Design review of the part built by this model. Coordinates are the model's own, in mm. A direction names the side the tool comes from. Coordinates: 2 decimals unless noted, no trailing zeros. Write each loop counter-clockwise with the first axis right and the second up, starting at its lowest first coordinate (ties: lowest second). Pieces come first, ordered by that corner, then holes. Notation, with made-up numbers: (-10, 86.5) - (1, 86.5) arc R10 ccw to (1, 91.5) - close; hole circle Ø9 at (70.5, 71). An arc over 180 degrees is marked (long way). Use a Markdown table: item, result.
from build123d import *

# Parameters (mm, degrees)
SKETCH1_R                = 205
SKETCH1_R_2              = 5
SKETCH1_R_3              = 175
BOSS_EXTRUDE1_DEPTH      = 2
BOSS_EXTRUDE2_DEPTH      = 7
BOSS_EXTRUDE2_DEPTH_BACK = 2
SKETCH2_R                = 207
SKETCH2_R_2              = 205
BOSS_EXTRUDE3_START      = 2
SKETCH3_R                = 207
SKETCH3_R_2              = 195
BOSS_EXTRUDE3_DEPTH      = 2


with BuildPart() as part:
    # Sketch1 → Boss-Extrude1 (new body)
    with BuildSketch(Plane(origin=(0, 0, 0), x_dir=(1, 0, 0), z_dir=(0, 1, 0))):
        with Locations(Location((0, 0, 0), (0, 0, 270))):
            Circle(SKETCH1_R)
        with Locations(Location((-185, 0, 0), (0, 0, 270))):
            Circle(SKETCH1_R_2, mode=Mode.SUBTRACT)
        with Locations(Location((0, 0, 0), (0, 0, 270))):
            Circle(SKETCH1_R_3, mode=Mode.SUBTRACT)
        with Locations(Location((-130.81475452, 130.81475452, 0), (0, 0, 270))):
            Circle(SKETCH1_R_2, mode=Mode.SUBTRACT)
        with Locations(Location((0, 185, 0), (0, 0, 270))):
            Circle(SKETCH1_R_2, mode=Mode.SUBTRACT)
        with Locations(Location((130.81475452, 130.81475452, 0), (0, 0, 270))):
            Circle(SKETCH1_R_2, mode=Mode.SUBTRACT)
        with Locations(Location((185, 0, 0), (0, 0, 270))):
            Circle(SKETCH1_R_2, mode=Mode.SUBTRACT)
        with Locations(Location((130.81475452, -130.81475452, 0), (0, 0, 270))):
            Circle(SKETCH1_R_2, mode=Mode.SUBTRACT)
        with Locations(Location((0, -185, 0), (0, 0, 270))):
            Circle(SKETCH1_R_2, mode=Mode.SUBTRACT)
        with Locations(Location((-130.81475452, -130.81475452, 0), (0, 0, 270))):
            Circle(SKETCH1_R_2, mode=Mode.SUBTRACT)
    extrude(amount=BOSS_EXTRUDE1_DEPTH)

    # Sketch2 → Boss-Extrude2 (add, two sides: drawn at the far end of the back side and taken through both)
    with BuildSketch(Plane.XZ.offset(-BOSS_EXTRUDE2_DEPTH_BACK)):
        with Locations(Location((0, 0, 0), (0, 0, 270))):
            Circle(SKETCH2_R)
        with Locations(Location((0, 0, 0), (0, 0, 270))):
            Circle(SKETCH2_R_2, mode=Mode.SUBTRACT)
    extrude(amount=BOSS_EXTRUDE2_DEPTH + BOSS_EXTRUDE2_DEPTH_BACK)

    # Sketch3 → Boss-Extrude3 (add)
    with BuildSketch(Plane.XZ.offset(7).offset(BOSS_EXTRUDE3_START)):
        with Locations(Location((0, 0, 0), (0, 0, 270))):
            Circle(SKETCH3_R)
        with Locations(Location((0, 0, 0), (0, 0, 270))):
            Circle(SKETCH3_R_2, mode=Mode.SUBTRACT)
    extrude(amount=-BOSS_EXTRUDE3_DEPTH)


solid = part.part
(1) Take a section at B-B on z = 0. Write out the cut boundary in (x, y), and give its area (3 significant figures).
Determined:
| item | result |
|---|---|
| outline | (-207, -9) - (-195, -9) - (-195, -7) - (-205, -7) - (-205, 0) - (-190, 0) - (-190, 2) - (-207, 2) - close; (-180, 0) - (-175, 0) - (-175, 2) - (-180, 2) - close; (175, 0) - (180, 0) - (180, 2) - (175, 2) - close; (190, 0) - (205, 0) - (205, -7) - (195, -7) - (195, -9) - (207, -9) - (207, 2) - (190, 2) - close |
| area | 164 mm2 |
(2) Machinability: for faces 5 (the cylindrical face through (189.957, 0.986, -0.651)), 6 (the flat face through (-75, -7, -181)), 7 (the cylindrical face through (-173, -8.01, -89.98)), which of the approach directions +Z, -Z, +X, -X, +Y, -Y give a long, thin tool a straight path to every point of the face, cutting with its end or side? Answer none if there is none.
Determined:
| item | result |
|---|---|
| face 5 | +Y, -Y |
| face 6 | none |
| face 7 | -Y |
(3) For L1, parallel to X at y = 0.85, z = 0; L2, parallel to Z at x = 6, y = -2.5; L3, parallel to Z at x = -122, y = -3.5, list the stretches that pass through material, from the lowest coordinate up. Write a range as from..to.
Determined:
| item | result |
|---|---|
| L1 | -207..-190, -180..-175, 175..180, 190..207 |
| L2 | -206.91..-204.91, 204.91..206.91 |
| L3 | -167.23..-164.75, 164.75..167.23 |
(4) Take a section at D-D on y = -3.5. Write out the cut boundary in (x, z).
Determined:
| item | result |
|---|---|
| outline | circle Ø414 at (0, 0); hole circle Ø410 at (0, 0) |
(5) Take a section at A-A on x = 0. Write out the cut boundary in (y, z).
Determined:
| item | result |
|---|---|
| outline | (-9, -207) - (2, -207) - (2, -190) - (0, -190) - (0, -205) - (-7, -205) - (-7, -195) - (-9, -195) - close; (-9, 195) - (-7, 195) - (-7, 205) - (0, 205) - (0, 190) - (2, 190) - (2, 207) - (-9, 207) - close; (0, -180) - (2, -180) - (2, -175) - (0, -175) - close; (0, 175) - (2, 175) - (2, 180) - (0, 180) - close |
(6) Draft analysis for pull direction Y (two halves, no side actions). For faces 1 (the cylindrical face through (-130.59, 0.99, -135.81)), 2 (the flat face through (-151, 0, 90)), 3 (the flat face through (-137, -9, 139)), 4 (the cylindrical face through (-200.125, -3.451, 44.44)), state which applies: +Y half, -Y half, draft (parallel to the pull), parting line (faces both ways), or undercut.
Determined:
| item | result |
|---|---|
| face 1 | draft |
| face 2 | undercut |
| face 3 | -Y half |
| face 4 | undercut |
(7) For pin 1 (9 mm diameter, centred on x = 185, z = 0, fed in from +Y); pin 2 (4 mm diameter, centred on x = -139.5, y = -5, fed in from -Z); pin 3 (3 mm diameter, centred on y = -6, z = -44.5, fed in from +X); pin 4 (16 mm diameter, centred on x = -185, z = 0, fed in from -Y), all flat-tipped, find the tip position at first contact; note any pin that passes through.
Determined:
| item | result |
|---|---|
| pin 1 | through |
| pin 2 | z = -154.73 |
| pin 3 | x = 202.48 |
| pin 4 | y = 0 |
(8) Take a section at C-C on x = 185. Write out the cut boundary in (y, z), and give its area (3 significant figures).
Determined:
| item | result |
|---|---|
| outline | (-9, -92.87) - (2, -92.87) - (2, -5) - (0, -5) - (0, -88.32) - (-7, -88.32) - (-7, -61.64) - (-9, -61.64) - close; (-9, 61.64) - (-7, 61.64) - (-7, 88.32) - (0, 88.32) - (0, 5) - (2, 5) - (2, 92.87) - (-9, 92.87) - close |
| area | 540 mm2 |
